The model under review builds one solid part; all positions refer to its coordinate system, in mm. Coordinates: 2 decimals unless noted, no trailing zeros. Order: outer loops, then holes, each group sorted by start corner. A loop starts at its lowest first (then second) coordinate and runs counter-clockwise, first axis right, second up. Notation, with made-up numbers: (-34, -35) -> (-18, -35) arc R7 cw to (-18, -30) -> close; hole circle Ø3 at (70, -18). An arc over 180 degrees is marked (long way). Use one line per item in the form item = value.
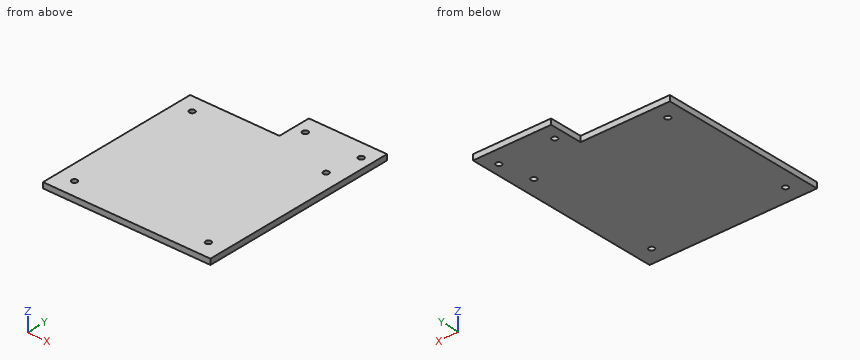
from build123d import *

# Parameters (mm, degrees)
SKETCH_1_R          = 5
EXTRUDE_1_DEPTH     = 10
SKETCH_3_W          = 10
SKETCH_3_H          = 60
EXTRUDE_2_DEPTH     = 40
CUT_EXTRUDE_2_DEPTH = 40


with BuildPart() as part:
    # Sketch 1 → Extrude 1 (new body)
    with BuildSketch(Plane.XY):
        Polygon((300, 360), (200, 360), (200, 300), (0, 300), (0, 0), (300, 0), (300, 300), align=None)
        with Locations((270, 30)):
            Circle(SKETCH_1_R, mode=Mode.SUBTRACT)
        with Locations((30, 30)):
            Circle(SKETCH_1_R, mode=Mode.SUBTRACT)
        with Locations((270, 270)):
            Circle(SKETCH_1_R, mode=Mode.SUBTRACT)
        with Locations((30, 270)):
            Circle(SKETCH_1_R, mode=Mode.SUBTRACT)
    extrude(amount=EXTRUDE_1_DEPTH)

    # Sketch 3 → Extrude 2 (add)
    with BuildSketch(Plane.ZY.offset(-200)):
        with Locations((5, 330)):
            Rectangle(SKETCH_3_W, SKETCH_3_H)
    extrude(amount=EXTRUDE_2_DEPTH)

    # Sketch 4 → Cut-Extrude 2 (cut)
    with BuildSketch(Plane.XY.offset(10)):
        with BuildLine():
            ThreePointArc((175, 330), (180, 325), (185, 330))
            Line((185, 330), (175, 330))
        make_face()
        with BuildLine():
            Line((175, 330), (185, 330))
            ThreePointArc((185, 330), (180, 335), (175, 330))
        make_face()
        with BuildLine():
            ThreePointArc((285, 330), (280, 335), (275, 330))
            Line((275, 330), (280, 330))
            Line((280, 330), (285, 330))
        make_face()
        with BuildLine():
            Line((280, 330), (275, 330))
            ThreePointArc((275, 330), (280, 325), (285, 330))
            Line((285, 330), (280, 330))
        make_face()
    extrude(amount=-CUT_EXTRUDE_2_DEPTH, mode=Mode.SUBTRACT)


solid = part.part
Item 1: Clearance check with flat-ended pins moving along their axes: pin 1 (9 mm diameter, centred on x = 270, y = 30, fed in from +Z); pin 2 (5 mm diameter, centred on x = 94, z = 6.5, fed in from +Y). State where each tip first meets the part, or that it passes through.
Results found:
pin_1 = through
pin_2 = 300
Item 2: To check wall thickness, follow L1, parallel to Y at x = 30, z = 2.25; L2, parallel to Y at x = 270, z = 2.5. State the ranges of each line that lie inside material, in increasing order. Write a range as from..to.
Results found:
L1 = 0..25, 35..265, 275..300
L2 = 0..25, 35..265, 275..360
Item 3: We need section D-D (x = 144). Write out the cut boundary in (y, z).
Results found:
outline = (0, 0) -> (300, 0) -> (300, 10) -> (0, 10) -> close
Item 4: We need section B-B (x = 270). Write out the cut boundary in (y, z).
Results found:
outline = (0, 0) -> (25, 0) -> (25, 10) -> (0, 10) -> close; (35, 0) -> (265, 0) -> (265, 10) -> (35, 10) -> close; (275, 0) -> (360, 0) -> (360, 10) -> (275, 10) -> close
Item 5: We need section C-C (z = 8.25). Write out the cut boundary in (x, y).
Results found:
outline = (0, 0) -> (300, 0) -> (300, 360) -> (160, 360) -> (160, 300) -> (0, 300) -> close; hole circle Ø10 at (30, 30); hole circle Ø10 at (30, 270); hole circle Ø10 at (180, 330); hole circle Ø10 at (270, 30); hole circle Ø10 at (270, 270); hole circle Ø10 at (280, 330)
Item 6: We need section A-A (y = 30). Write out the cut boundary in (x, z).
Results found:
outline = (0, 0) -> (25, 0) -> (25, 10) -> (0, 10) -> close; (35, 0) -> (265, 0) -> (265, 10) -> (35, 10) -> close; (275, 0) -> (300, 0) -> (300, 10) -> (275, 10) -> close
